Part model, mm, in its own coordinate system. Face numbers are marked on the shaded views. A direction names the side the tool comes from. Round coordinates to 2 decimals unless told otherwise and drop trailing zeros. Write each loop counter-clockwise with the first axis right and the second up, starting at its lowest first coordinate (ties: lowest second). Pieces come first, ordered by that corner, then holes. Notation, with made-up numbers: (-17.5, 79) -> (-3.5, 79) arc R22 ccw to (-3.5, 106) -> close; hole circle Ø11 at (51, 72.25). An arc over 180 degrees is marked (long way). Return JSON: item names as keys, results as strings. Group by question number.
(1) Mould opens along X. For the marked faces 1, 2 and 3 say: +X half, -X half, draft (parallel to the pull), parting line (faces both ways), or undercut.
(2) Saw through at C-C (y = 24). List the corners of the cut face in (x, z).
(3) Saw through at B-B (x = -20.5). List the corners of the cut face in (y, z), plus the area to 3 significant figures.
(4) Drill centre lines: L1, parallel to Y at x = -37.5, z = 80.5; L2, parallel to Z at x = -23, y = 68; L3, parallel to Z at x = 18.5, y = 4.5. Where is each one in solid material? Low to high. Write a range as from..to.
(5) Tool access for the marked faces 4, 5, 6, 7 and 8: list every direction of +Z, -Z, +X, -X, +Y, -Y with a clear straight run to the whole face (end or side of a thin tool).
(6) Saw through at D-D (y = 70). List the corners of the cut face in (x, z), plus the area to 3 significant figures.
(7) Drop flat-ended pins along their axis: pin 1 Ø10 at (y, z) = (15.5, 26) entering from +X; pin 2 Ø10 at (x, z) = (7, 47) entering from -Y; pin 3 Ø18 at (x, y) = (50.5, 23.5) entering from +Z. Give the stop position or say it passes through.
(8) Saw through at A-A (z = 67). List the corners of the cut face in (x, y), plus the area to 3 significant figures.
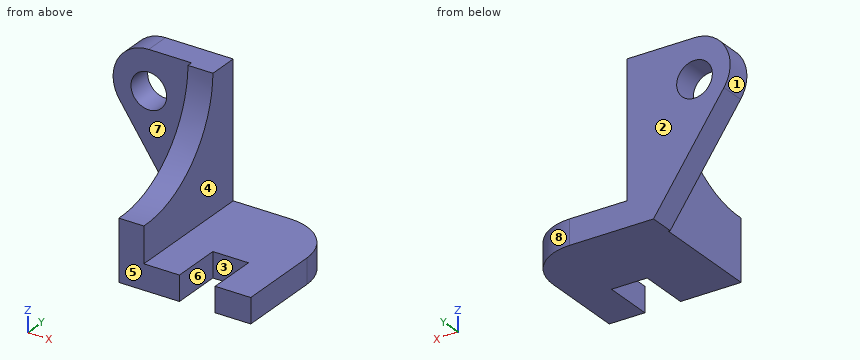
from build123d import *

# Parameters (mm, degrees)
BASE_PLATE_14MM_DEPTH  = 14
UPRIGHT_START          = 1
UPRIGHT_WEB_14MM_DEPTH = 14
SIDE_LUG_SKETCH_R      = 10
SIDE_LUG_14MM_DEPTH    = 14
CORNER_ROUND_R28_R     = 28


with BuildPart() as part:
    # Base Plate Sketch → Base Plate 14mm (new body)
    with BuildSketch(Plane.XY):
        Polygon((1, 0), (1, 75), (75, 75), (75, 0), (55, 0), (55, 28), (35, 28), (35, 0), align=None)
    extrude(amount=BASE_PLATE_14MM_DEPTH)

    # Upright Web Sketch → Upright Web 14mm (add)
    with BuildSketch(Plane(origin=(0, 0, 0), x_dir=(0, 0, -1), z_dir=(1, 0, 0)).offset(UPRIGHT_START)):
        with BuildLine():
            Line((-14, 75), (-89, 75))
            Line((-89, 75), (-89, 58))
            ThreePointArc((-89, 58), (-49.329041508, 40.541426156), (-34, 0))
            Line((-34, 0), (-14, 0))
            Line((-14, 0), (-14, 75))
        make_face()
    extrude(amount=UPRIGHT_WEB_14MM_DEPTH)

    # Side Lug Sketch → Side Lug 14mm (add)
    with BuildSketch(Plane(origin=(0, 75, 0), x_dir=(1, 0, 0), z_dir=(0, 1, 0))):
        with BuildLine():
            Line((1, -89), (-23, -89))
            ThreePointArc((-23, -89), (-40.691278494, -78.328379563), (-39.503096073, -57.701866526))
            Line((-39.503096073, -57.701866526), (0, 0))
            Line((0, 0), (1, 0))
            Line((1, 0), (1, -89))
        make_face()
        with Locations(Location((-23, -67, 0), (0, 0, 180))):
            Circle(SIDE_LUG_SKETCH_R, mode=Mode.SUBTRACT)
    extrude(amount=-SIDE_LUG_14MM_DEPTH)

    # Corner Round R28
    corner_round_r28_edges = [part.edges().sort_by_distance(p)[0] for p in [
        (75, 75, 7),
    ]]
    fillet(corner_round_r28_edges, radius=CORNER_ROUND_R28_R)


solid = part.part
Computed values:
{
 "1": {"face 1": "-X half", "face 2": "draft", "face 3": "undercut"},
 "2": {"outline": "(1, 0) -> (35, 0) -> (35, 14) -> (15, 14) -> (15, 38.46) -> (1, 38.46) -> close; (55, 0) -> (75, 0) -> (75, 14) -> (55, 14) -> close"},
 "3": {"outline": "(61, 29.94) -> (75, 29.94) -> (75, 57.32) -> (61, 57.32) -> close; (61, 76.68) -> (75, 76.68) -> (75, 89) -> (61, 89) -> close", "area": "556 mm2"},
 "4": {"L1": "61..75", "L2": "33.6..57, 77..89", "L3": "0..14"},
 "5": {"face 4": "+Z, +X, +Y, -Y", "face 5": "+Z, -Z, +X, -X, -Y", "face 6": "+Z, -Z, -Y", "face 7": "+Z, -Z, -X, -Y", "face 8": "+Z, -Z, +X, +Y"},
 "6": {"outline": "(-39.5, 57.7) -> (0, 0) -> (62.97, 0) -> (62.97, 14) -> (15, 14) -> (15, 89) -> (-23, 89) arc R20 ccw to start; hole circle Ø20 at (-23, 67)", "area": "4,080 mm2"},
 "7": {"pin 1": "x = 15", "pin 2": "y = 30.91", "pin 3": "z = 14"},
 "8": {"outline": "(-42.9, 61) -> (-33, 61) -> (-33, 75) -> (-42.9, 75) -> close; (-13, 61) -> (1, 61) -> (1, 53.08) -> (15, 53.08) -> (15, 75) -> (-13, 75) -> close", "area": "641 mm2"}
}
